```python
from build123d import *

# Parameters (mm, degrees)
SKETCH1_W                                            = 260
SKETCH1_H                                            = 106
BOSS_EXTRUDE1_DEPTH                                  = 7.5
CUT_EXTRUDE1_DEPTH                                   = 142.187818171
CUT_EXTRUDE2_DEPTH                                   = 2
M6_TAPPED_HOLE1_D                                    = 5
SKETCH9_W                                            = 20
SKETCH9_H                                            = 40
CUT_EXTRUDE4_DEPTH                                   = 142.187818171
FILLET5_R                                            = 3
HOLE_SIZE_PER_SOCKET_HEAD_CAP_SCREW_TYPE_D           = 5.5
HOLE_SIZE_PER_SOCKET_HEAD_CAP_SCREW_TYPE_CBORE_D     = 10
HOLE_SIZE_PER_SOCKET_HEAD_CAP_SCREW_TYPE_CBORE_DEPTH = 6
CHAMFER1_SIZE                                        = 2
M3_TAPPED_HOLE1_D                                    = 2.5
M3_TAPPED_HOLE1_DEPTH                                = 7.5
M3_TAPPED_HOLE1_TIP                                  = 0.751075774
F_10_0_10_DIAMETER_HOLE1_D                           = 10


with BuildPart() as part:
    # Sketch1 → Boss-Extrude1 (new, symmetric)
    with BuildSketch(Plane(origin=(0, 0, 0), x_dir=(1, 0, 0), z_dir=(0, 1, 0))):
        Rectangle(SKETCH1_W, SKETCH1_H)
    extrude(amount=BOSS_EXTRUDE1_DEPTH, both=True)

    # Sketch2 → Cut-Extrude1 (cut, through all)
    with BuildSketch(Plane(origin=(0, 7.5, 0), x_dir=(1, 0, 0), z_dir=(0, 1, 0))):
        Polygon((55, 53), (-130, 53), (-130, 18), (-110, 18), align=None)
        Polygon((-130, -18), (-130, -53), (55, -53), (-110, -18), align=None)
    extrude(amount=-CUT_EXTRUDE1_DEPTH, mode=Mode.SUBTRACT)

    # Sketch3 → Cut-Extrude2 (cut)
    with BuildSketch(Plane(origin=(0, 7.5, 0), x_dir=(1, 0, 0), z_dir=(0, 1, 0))):
        with BuildLine():
            Line((-130, 4), (-77, 4))
            ThreePointArc((-77, 4), (-75.585786438, 3.414213562), (-75, 2))
            Line((-75, 2), (-75, -2))
            ThreePointArc((-75, -2), (-75.585786438, -3.414213562), (-77, -4))
            Line((-77, -4), (-130, -4))
            Line((-130, -4), (-130, 4))
        make_face()
    extrude(amount=-CUT_EXTRUDE2_DEPTH, mode=Mode.SUBTRACT)

    # M6 Tapped Hole1 (through all)
    with Locations(Plane(origin=(0, 7.5, 0), x_dir=(1, 0, 0), z_dir=(0, 1, 0))):
        with Locations((-99, 12), (-99, -12)):
            Hole(M6_TAPPED_HOLE1_D / 2)

    # Sketch9 → Cut-Extrude4 (cut, through all)
    with BuildSketch(Plane(origin=(0, 7.5, 0), x_dir=(1, 0, 0), z_dir=(0, 1, 0))):
        with Locations((45, 0)):
            Rectangle(SKETCH9_W, SKETCH9_H)
    extrude(amount=-CUT_EXTRUDE4_DEPTH, mode=Mode.SUBTRACT)

    # Fillet5
    fillet5_edges = [part.edges().sort_by_distance(p)[0] for p in [
        (55, 0, -20),
        (55, 0, 20),
        (35, 0, 20),
        (35, 0, -20),
    ]]
    fillet(fillet5_edges, radius=FILLET5_R)

    # Hole size per socket head cap screw type1 (through all)
    with Locations(Plane(origin=(0, -7.5, 0), x_dir=(-1, 0, 0), z_dir=(0, -1, 0))):
        with Locations((-122.5, -47), (-97.5, -47), (-72.5, -47), (-72.5, 47), (-97.5, 47), (-122.5, 47)):
            CounterBoreHole(HOLE_SIZE_PER_SOCKET_HEAD_CAP_SCREW_TYPE_D / 2, HOLE_SIZE_PER_SOCKET_HEAD_CAP_SCREW_TYPE_CBORE_D / 2, HOLE_SIZE_PER_SOCKET_HEAD_CAP_SCREW_TYPE_CBORE_DEPTH)

    # Chamfer1
    chamfer1_edges = [part.edges().sort_by_distance(p)[0] for p in [
        (-130, 0, -18),
        (-130, 0, 18),
    ]]
    chamfer(chamfer1_edges, length=CHAMFER1_SIZE)

    # M3 Tapped Hole1
    with Locations(Plane(origin=(0, 7.5, 0), x_dir=(1, 0, 0), z_dir=(0, 1, 0))):
        with Locations((40, 38), (-60, 18)):
            Hole(M3_TAPPED_HOLE1_D / 2, depth=M3_TAPPED_HOLE1_DEPTH)
            with Locations((0, 0, -(M3_TAPPED_HOLE1_DEPTH + M3_TAPPED_HOLE1_TIP / 2))):  # 118° drill point
                Cone(0, M3_TAPPED_HOLE1_D / 2, M3_TAPPED_HOLE1_TIP, mode=Mode.SUBTRACT)

    # Ø10.0 (10) Diameter Hole1 (through all)
    with Locations(Plane(origin=(0, 7.5, 0), x_dir=(1, 0, 0), z_dir=(0, 1, 0))):
        with Locations((-40, 20), (-40, -20), (20, -30), (20, 30)):
            Hole(F_10_0_10_DIAMETER_HOLE1_D / 2)


solid = part.part
```
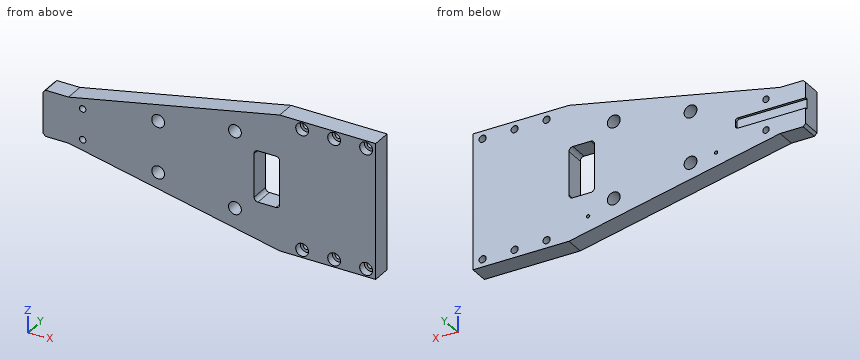
The model under review builds one solid part; all positions refer to its coordinate system, in mm. Round coordinates to 2 decimals unless told otherwise and drop trailing zeros. Order: outer loops, then holes, each group sorted by start corner. A loop starts at its lowest first (then second) coordinate and runs counter-clockwise, first axis right, second up. Notation, with made-up numbers: (-17, 29) - (11, 29) arc R21 cw to (11, 35) - close; hole circle Ø7 at (37, 2). An arc over 180 degrees is marked (long way). Answer in a Markdown table with one row per item.
(1) Take a section at D-D on x = -88. Write out the cut boundary in (y, z), plus the area to 3 significant figures.
Result set:
| item | result |
|---|---|
| outline | (-7.5, -22.67) - (7.5, -22.67) - (7.5, -4) - (5.5, -4) - (5.5, 4) - (7.5, 4) - (7.5, 22.67) - (-7.5, 22.67) - close |
| area | 664 mm2 |
(2) Take a section at A-A on x = 122.5. Write out the cut boundary in (y, z), plus the area to 3 significant figures.
Result set:
| item | result |
|---|---|
| outline | (-7.5, -53) - (7.5, -53) - (7.5, -49.75) - (-1.5, -49.75) - (-1.5, -52) - (-7.5, -52) - close; (-7.5, -42) - (-1.5, -42) - (-1.5, -44.25) - (7.5, -44.25) - (7.5, 44.25) - (-1.5, 44.25) - (-1.5, 42) - (-7.5, 42) - close; (-7.5, 52) - (-1.5, 52) - (-1.5, 49.75) - (7.5, 49.75) - (7.5, 53) - (-7.5, 53) - close |
| area | 1,370 mm2 |
(3) Take a section at B-B on z = 47. Write out the cut boundary in (x, y), plus the area to 3 significant figures.
Result set:
| item | result |
|---|---|
| outline | (26.71, -7.5) - (67.5, -7.5) - (67.5, -1.5) - (69.75, -1.5) - (69.75, 7.5) - (26.71, 7.5) - close; (75.25, -1.5) - (77.5, -1.5) - (77.5, -7.5) - (92.5, -7.5) - (92.5, -1.5) - (94.75, -1.5) - (94.75, 7.5) - (75.25, 7.5) - close; (100.25, -1.5) - (102.5, -1.5) - (102.5, -7.5) - (117.5, -7.5) - (117.5, -1.5) - (119.75, -1.5) - (119.75, 7.5) - (100.25, 7.5) - close; (125.25, -1.5) - (127.5, -1.5) - (127.5, -7.5) - (130, -7.5) - (130, 7.5) - (125.25, 7.5) - close |
| area | 1,220 mm2 |
(4) For line 1 (Z direction, x = 122.5, y = -5); line 2 (X direction, y = 2, z = -12); line 3 (Z direction, x = 122.5, y = 0.5), list the stretches that pass through material, from the lowest coordinate up. Write a range as from..to.
Result set:
| item | result |
|---|---|
| line 1 | z = -53..-52, -42..42, 52..53 |
| line 2 | x = -130..-101.5, -96.5..35, 55..130 |
| line 3 | z = -53..-49.75, -44.25..44.25, 49.75..53 |
(5) Take a section at C-C on x = -40. Write out the cut boundary in (y, z).
Result set:
| item | result |
|---|---|
| outline | (-7.5, -32.85) - (7.5, -32.85) - (7.5, -25) - (-7.5, -25) - close; (-7.5, -15) - (7.5, -15) - (7.5, 15) - (-7.5, 15) - close; (-7.5, 25) - (7.5, 25) - (7.5, 32.85) - (-7.5, 32.85) - close |
(6) Clearance check with flat-ended pins moving along their axes: P1, Ø6, axis at x = 46, y = 3, coming from the -Z side; P2, Ø7, axis at x = 72.5, z = -47, coming from the -Y side; P3, Ø0.6, axis at x = -102.5, y = 6.5, coming from the -Z side. State where each tip first meets the part, or that it passes through.
Result set:
| item | result |
|---|---|
| P1 | stops at z = -51.73 |
| P2 | stops at y = -1.5 |
| P3 | stops at z = -19.65 |
